The model under review builds one solid part; all positions refer to its coordinate system, in mm. A direction names the side the tool comes from. Coordinates: 2 decimals unless noted, no trailing zeros. Order: outer loops, then holes, each group sorted by start corner. A loop starts at its lowest first (then second) coordinate and runs counter-clockwise, first axis right, second up. Notation, with made-up numbers: (83.5, -26.75) -> (134.5, -26.75) arc R17 ccw to (134.5, -0.75) -> close; hole circle Ø6 at (-27, 83). An arc over 180 degrees is marked (long way). Use one line per item in the form item = value.
from build123d import *

# Parameters (mm, degrees)
CUT_EXTRUDE_1_DEPTH = 3


with BuildPart() as part:
    # 草图1 → 旋转1 (revolve)
    with BuildSketch(Plane.XY, mode=Mode.PRIVATE) as revolve_1_sk:
        Polygon((-6, 0), (-6, 4.4), (-5.4, 5), (0, 5), (0, 3), (15.3865, 3), (16, 2.3865), (16, 0), align=None)
    revolve(revolve_1_sk.sketch.rotate(Axis((16, 0, 0), (-1, 0, 0)), 270), axis=Axis((16, 0, 0), (-1, 0, 0)))

    # 草图2 → 切除-旋转1 (revolve, cut)
    with BuildSketch(Plane.XY, mode=Mode.PRIVATE) as cut_revolve_1_sk:
        Polygon((-6, 0), (-6, 2.5), (-3, 2.5), (-2.330127019, 0), align=None)
    revolve(cut_revolve_1_sk.sketch.rotate(Axis((-2.330127019, 0, 0), (-1, 0, 0)), 270), axis=Axis((-2.330127019, 0, 0), (-1, 0, 0)), mode=Mode.SUBTRACT)

    # 草图3 → 切除-拉伸1 (cut)
    with BuildSketch(Plane(origin=(-6, 0, 0), x_dir=(0, 0, -1), z_dir=(1, 0, 0))):
        Polygon((-2.5, 1.443375673), (-2.5, -1.443375673), (0, -2.886751346), (2.5, -1.443375673), (2.5, 1.443375673), (0, 2.886751346), align=None)
    extrude(amount=CUT_EXTRUDE_1_DEPTH, mode=Mode.SUBTRACT)


solid = part.part
Item 1: To check wall thickness, follow L1, parallel to X at y = -3.5, z = 0.75; L2, parallel to Y at x = -3.5, z = -4.5; L3, parallel to Y at x = -4.25, z = -0.5. State the ranges of each line that lie inside material, in increasing order. Write a range as from..to.
Results found:
L1 = -6..0
L2 = -2.18..2.18
L3 = -4.97..-2.6, 2.6..4.97
Item 2: Tool access review of faces 1 (the face through (-2.66, -4.88, -1.08)), 2 (the face through (0, -3.3, -0.1)), 3 (the face through (-4.521, 2.175, 1.233)): name each direction out of +Z, -Z, +X, -X, +Y, -Y from which nothing blocks a thin tool from reaching the whole face with its end or side.
Results found:
face_1 = +X, -X
face_2 = +X
face_3 = -X
Item 3: Clearance check with flat-ended pins moving along their axes: pin 1 (6 mm diameter, centred on y = 3, z = 3.5, fed in from +X); pin 2 (3 mm diameter, centred on x = -3, y = 2, fed in from -Z); pin 3 (4 mm diameter, centred on x = -0.5, z = 4, fed in from +Y); pin 4 (0.6 mm diameter, centred on y = 0.5, z = -1.5, fed in from -X). State where each tip first meets the part, or that it passes through.
Results found:
pin_1 = 16
pin_2 = -4.97
pin_3 = 4.58
pin_4 = -2.83
Item 4: We need section A-A (x = 0.5). Write out the cut boundary in (y, z), plus the area to 3 significant figures.
Results found:
outline = circle Ø6 at (0, 0)
area = 28.3 mm²
Item 5: Draft analysis for pull direction Y (two halves, no side actions). For faces 4 (the face through (16, 0, 0)), 5 (the face through (7.8, 0.9, 2.86)), 6 (the face through (-2.363, -0.074, -0.096)), 7 (the face through (-4.521, 2.155, -1.267)), state which applies: released by +Y, released by -Y, zero draft, split by the parting line, or undercut.
Results found:
face_4 = zero draft
face_5 = split by the parting line
face_6 = undercut
face_7 = undercut
